```python
from build123d import *

# Parameters (mm, degrees)
SKETCH_1_W                  = 25
SKETCH_1_H                  = 110
EXTRUDE_1_DEPTH             = 10
CHAMFER_1_SIZE              = 2
HOLE_WIZARD_1_D             = 5.5
HOLE_WIZARD_1_DEPTH         = 12.4
HOLE_WIZARD_1_CBORE_D       = 10
HOLE_WIZARD_1_CBORE_DEPTH   = 5.7
HOLE_WIZARD_1_TIP           = 1.652366702
HOLE_WIZARD_1_2_D           = 3.4
HOLE_WIZARD_1_2_DEPTH       = 15
HOLE_WIZARD_1_2_CBORE_D     = 6
HOLE_WIZARD_1_2_CBORE_DEPTH = 3.4
HOLE_WIZARD_1_2_TIP         = 1.021463052
SKETCH_6_R                  = 2.5
CUT_EXTRUDE_1_DEPTH         = 3.5


with BuildPart() as part:
    # 草图1 → 凸台-拉伸1 (new body)
    with BuildSketch(Plane(origin=(0, 0, 0), x_dir=(1, 0, 0), z_dir=(0, 1, 0))):
        Rectangle(SKETCH_1_W, SKETCH_1_H)
    extrude(amount=EXTRUDE_1_DEPTH)

    # 倒角1
    chamfer_1_edges = [part.edges().sort_by_distance(p)[0] for p in [
        (12.5, 5, 55),
        (-12.5, 5, 55),
        (-12.5, 5, -55),
        (12.5, 5, -55),
    ]]
    chamfer(chamfer_1_edges, length=CHAMFER_1_SIZE)

    # Hole Wizard 1
    with Locations(Plane(origin=(0, 10, 0), x_dir=(1, 0, 0), z_dir=(0, 1, 0))):
        with Locations((-6.5, -45), (-6.5, 0), (-6.5, 45), (-6.5, -22.5), (-6.5, 22.5)):
            CounterBoreHole(HOLE_WIZARD_1_D / 2, HOLE_WIZARD_1_CBORE_D / 2, HOLE_WIZARD_1_CBORE_DEPTH, depth=HOLE_WIZARD_1_DEPTH)
            with Locations((0, 0, -(HOLE_WIZARD_1_DEPTH + HOLE_WIZARD_1_TIP / 2))):  # 118° drill point
                Cone(0, HOLE_WIZARD_1_D / 2, HOLE_WIZARD_1_TIP, mode=Mode.SUBTRACT)

    # Hole Wizard 1 2
    with Locations(Plane(origin=(0, 0, 0), x_dir=(-1, 0, 0), z_dir=(0, -1, 0))):
        with Locations((-2.5, -36), (-2.5, 36)):
            CounterBoreHole(HOLE_WIZARD_1_2_D / 2, HOLE_WIZARD_1_2_CBORE_D / 2, HOLE_WIZARD_1_2_CBORE_DEPTH, depth=HOLE_WIZARD_1_2_DEPTH)
            with Locations((0, 0, -(HOLE_WIZARD_1_2_DEPTH + HOLE_WIZARD_1_2_TIP / 2))):  # 118° drill point
                Cone(0, HOLE_WIZARD_1_2_D / 2, HOLE_WIZARD_1_2_TIP, mode=Mode.SUBTRACT)

    # 草图6 → 切除-拉伸1 (cut)
    with BuildSketch(Plane(origin=(0, 10, 0), x_dir=(1, 0, 0), z_dir=(0, 1, 0))):
        with Locations(Location((2.5, -36, 0), (0, 0, 270))):
            Circle(SKETCH_6_R)
        with Locations(Location((2.5, 36, 0), (0, 0, 270))):
            Circle(SKETCH_6_R)
    extrude(amount=-CUT_EXTRUDE_1_DEPTH, mode=Mode.SUBTRACT)


solid = part.part
```
Check sheet for the modelled part. Datum: model origin and axes. Units: mm. A direction names the side the tool comes from. Round coordinates to 2 decimals unless told otherwise and drop trailing zeros. Order: outer loops, then holes, each group sorted by start corner. A loop starts at its lowest first (then second) coordinate and runs counter-clockwise, first axis right, second up. Notation, with made-up numbers: (78, -8) - (123, -8) arc R26 ccw to (123, 16) - close; hole circle Ø10 at (86, -37). An arc over 180 degrees is marked (long way). Answer as CSV lines item,"result". Start each with the question number.
1) Depth check by flat-ended pin: pin 1 (4.5 mm diameter, centred on x = -6.5, z = 22.5, fed in from -Y); pin 2 (2.5 mm diameter, centred on x = 3, z = -36.5, fed in from +Y); pin 3 (5 mm diameter, centred on x = -7.5, z = -46.5, fed in from +Y); pin 4 (5 mm diameter, centred on x = 2.5, z = -36, fed in from -Y). Enter the tip coordinate at first touch or a pass-through.
2) Section check A-A (z = -36). Record the cut outline in (x, y), then the cut area to 3 significant figures.
3) Section check B-B (x = 2.5). Record the cut outline in (y, z), then the cut area to 3 significant figures.
4) Section check C-C (z = 0). Record the cut outline in (x, y), then the cut area to 3 significant figures.
5) Scan lines: probe 1 along Z at (x, y) = (-6.5, 8.6); probe 2 along Z at (x, y) = (2.5, 4.15); probe 3 along Z at (x, y) = (2.5, 2.6). Record each from-to range of solid material in increasing order.
6) Section check D-D (x = -6.5). Give the number of separate pieces and of enclosed holes in the cut face, then the cut area to 3 significant figures.
7) Draft check along Z on faces 1 (the face through (0, 5, 55)), 2 (the face through (2.891, 1.676, -38.974)), 3 (the face through (0, 0, -1)). Enter one of: +Z half, -Z half, draft (parallel to the pull), parting line (faces both ways), or undercut.
8) Tool access check on faces 4 (the face through (3.3, 5, 37.5)), 5 (the face through (-4, 4.3, 25)), 6 (the face through (2.891, 1.676, 33.026)). Record the directions out of +Z, -Z, +X, -X, +Y, -Y that give a thin tool (end or side, any length) a straight path to the whole face; none if there is none.
Determined:
1,pin 1,"through"
1,pin 2,"y = 6.5"
1,pin 3,"y = 4.3"
1,pin 4,"y = 3.4"
2,outline,"(-12.5, 0) - (-0.5, 0) - (-0.5, 3.4) - (0.8, 3.4) - (0.8, 6.5) - (0, 6.5) - (0, 10) - (-12.5, 10) - close; (4.2, 3.4) - (5.5, 3.4) - (5.5, 0) - (12.5, 0) - (12.5, 10) - (5, 10) - (5, 6.5) - (4.2, 6.5) - close"
2,area,"202 mm^2"
3,outline,"(0, -55) - (10, -55) - (10, -38.5) - (6.5, -38.5) - (6.5, -37.7) - (3.4, -37.7) - (3.4, -39) - (0, -39) - close; (0, -33) - (3.4, -33) - (3.4, -34.3) - (6.5, -34.3) - (6.5, -33.5) - (10, -33.5) - (10, 33.5) - (6.5, 33.5) - (6.5, 34.3) - (3.4, 34.3) - (3.4, 33) - (0, 33) - close; (0, 39) - (3.4, 39) - (3.4, 37.7) - (6.5, 37.7) - (6.5, 38.5) - (10, 38.5) - (10, 55) - (0, 55) - close"
3,area,"1,000 mm^2"
4,outline,"(-12.5, 0) - (-9.25, 0) - (-9.25, 4.3) - (-11.5, 4.3) - (-11.5, 10) - (-12.5, 10) - close; (-3.75, 0) - (12.5, 0) - (12.5, 10) - (-1.5, 10) - (-1.5, 4.3) - (-3.75, 4.3) - close"
4,area,"169 mm^2"
5,probe 1,"-55 to -50, -40 to -27.5, -17.5 to -5, 5 to 17.5, 27.5 to 40, 50 to 55"
5,probe 2,"-55 to -37.7, -34.3 to 34.3, 37.7 to 55"
5,probe 3,"-55 to -39, -33 to 33, 39 to 55"
6,separate pieces,"6"
6,enclosed holes,"0"
6,area,"697 mm^2"
7,face 1,"+Z half"
7,face 2,"undercut"
7,face 3,"draft"
8,face 4,"+Y, -Y"
8,face 5,"+Y"
8,face 6,"-Y"
